from build123d import *

# Parameters (mm, degrees)
M3_TAPPED_HOLE1_D    = 2.5
SKETCH3_OUTSIDE_W    = 37.982
SKETCH3_OUTSIDE_H    = 37.982
SKETCH3_OUTSIDE_R    = 9.25
CUT_EXTRUDE2_DEPTH   = 1
M3_CLEARANCE_HOLE1_D = 3.4
SKETCH6_W            = 10
SKETCH6_H            = 31.428384658
CUT_EXTRUDE3_DEPTH   = 1
M4_TAPPED_HOLE1_D    = 3.3
CHAMFER1_SIZE        = 0.5
CHAMFER2_SIZE        = 0.2


with BuildPart() as part:
    # Sketch1 → Revolve1 (revolve)
    with BuildSketch(Plane.XY, mode=Mode.PRIVATE) as revolve1_sk:
        Polygon((4.5, 5), (6, 5), (14, 5), (14, 0), (0, 0), (0, 5), align=None)
    revolve(revolve1_sk.sketch.rotate(Axis((0, 0, 0), (0, 1, 0)), 90), axis=Axis((0, 0, 0), (0, 1, 0)))

    # M3 Tapped Hole1 (through all)
    with Locations(Plane(origin=(0, 5, 0), x_dir=(1, 0, 0), z_dir=(0, 1, 0))):
        with Locations((-6.5, 0), (6.5, 0)):
            Hole(M3_TAPPED_HOLE1_D / 2)

    # Sketch3 outside → Cut-Extrude2 (cut)
    with BuildSketch(Plane(origin=(0, 5, 0), x_dir=(1, 0, 0), z_dir=(0, 1, 0))):
        Rectangle(SKETCH3_OUTSIDE_W, SKETCH3_OUTSIDE_H)
        with Locations(Location((0, 0, 0), (0, 0, 270))):
            Circle(SKETCH3_OUTSIDE_R, mode=Mode.SUBTRACT)
    extrude(amount=-CUT_EXTRUDE2_DEPTH, mode=Mode.SUBTRACT)

    # M3 Clearance Hole1 (through all)
    with Locations(Plane(origin=(0, 0, 0), x_dir=(-1, 0, 0), z_dir=(0, -1, 0))):
        with Locations((10, -6), (10, 6), (-10, -6), (-10, 6)):
            Hole(M3_CLEARANCE_HOLE1_D / 2)

    # Sketch6 → Cut-Extrude3 (cut)
    with BuildSketch(Plane.XZ):
        Rectangle(SKETCH6_W, SKETCH6_H)
    extrude(amount=-CUT_EXTRUDE3_DEPTH, mode=Mode.SUBTRACT)

    # M4 Tapped Hole1 (through all)
    with Locations(Plane(origin=(0, 1, 0), x_dir=(-1, 0, 0), z_dir=(0, -1, 0))):
        with Locations((0, 0)):
            Hole(M4_TAPPED_HOLE1_D / 2)

    # Chamfer1
    chamfer1_edges = [part.edges().sort_by_distance(p)[0] for p in [
        (0, 4, 14),
        (14, 0, 0),
        (-14, 0, 0),
    ]]
    chamfer(chamfer1_edges, length=CHAMFER1_SIZE)

    # Chamfer2
    chamfer2_edges = [part.edges().sort_by_distance(p)[0] for p in [
        (0, 5, -9.25),
    ]]
    chamfer(chamfer2_edges, length=CHAMFER2_SIZE)


solid = part.part
Can you work these out from the model? Positions are in its coordinate system, mm. A direction names the side the tool comes from. Coordinates: 2 decimals unless noted, no trailing zeros. Order: outer loops, then holes, each group sorted by start corner. A loop starts at its lowest first (then second) coordinate and runs counter-clockwise, first axis right, second up. Notation, with made-up numbers: M 55,77.5 L 84,77.5 A19 ccw 84,97.5 Z; hole C 69.5,-33.5 d9. An arc over 180 degrees is marked long. Write item = value, one per line.
(1) For pin 1 Ø3 at (x, z) = (7.5, 9) entering from +Y; pin 2 Ø1.5 at (y, z) = (4, -3) entering from -X; pin 3 Ø0.5 at (y, z) = (0.5, 0.5) entering from +X, each with a flat end and sliding along its axis, tell me the tip position at first contact or that it passes through.
Results are:
pin_1 = 4
pin_2 = -13.79
pin_3 = 14
(2) Suppose I cut it at D-D on x = -10. State how many separate pieces and enclosed holes the cut face has, plus the area to 3 significant figures.
Results are:
separate_pieces = 3
enclosed_holes = 0
area = 50.5 mm2
(3) Suppose I cut it at C-C on y = 4.4. Please give me the cut outline in (x, z).
Results are:
outline = C 0,0 d18.5; hole C -6.5,0 d2.5; hole C 0,0 d3.3; hole C 6.5,0 d2.5
(4) I need wall thicknesses on line 1 along Z through (x, y) = (-10, 2.5); line 2 along Y through (x, z) = (12.25, 3.5); line 3 along X through (y, z) = (1.7, 6). Which ranges of each line are inside material? Lowest first, please. Write a range as [from, to].
Results are:
line_1 = [-9.8, -7.7], [-4.3, 4.3], [7.7, 9.8]
line_2 = [0, 4]
line_3 = [-12.65, -11.7], [-8.3, 8.3], [11.7, 12.65]
(5) If we mould it in two halves opening along X, with no side actions, what happens to faces 1 (the face through (-13.64, 0.14, -0.23)), 2 (the face through (13.64, 0.14, 0.23)), 3 (the face through (7.75, 2.46, -0.05))? For each: pulls with the +X half, pulls with the -X half, needs draft (parallel to the pull), parting line crosses it, or undercut.
Results are:
face_1 = pulls with the -X half
face_2 = pulls with the +X half
face_3 = undercut
(6) Suppose I cut it at B-B on y = 2.4. Please give me the cut outline in (x, z), plus the area to 3 significant figures.
Results are:
outline = C 0,0 d28; hole C -10,-6 d3.4; hole C -10,6 d3.4; hole C -6.5,0 d2.5; hole C 0,0 d3.3; hole C 6.5,0 d2.5; hole C 10,-6 d3.4; hole C 10,6 d3.4
area = 561 mm2
(7) Suppose I cut it at A-A on x = 0. Please give me the cut outline in (y, z), plus the area to 3 significant figures.
Results are:
outline = M 1,-14 L 3.5,-14 L 4,-13.5 L 4,-9.25 L 4.8,-9.25 L 5,-9.05 L 5,-1.65 L 1,-1.65 Z; M 1,1.65 L 5,1.65 L 5,9.05 L 4.8,9.25 L 4,9.25 L 4,13.5 L 3.5,14 L 1,14 Z
area = 89.0 mm2
(8) For faces 4 (the face through (-5, 0.5, -0.2)), 5 (the face through (13.67, 1.98, 3.03)), 6 (the face through (-3.543, 4.406, 8.545)), which set-ups out of +Z, -Z, +X, -X, +Y, -Y let a thin tool reach every point of the face, with its end or its side?
Results are:
face_4 = +Z, -Z, -Y
face_5 = +Y, -Y
face_6 = +Y
